The listing builds one solid part. Answer for the finished solid, in the listing's coordinates (mm). A direction names the side the tool comes from. Give positions to 0.01 mm unless a question says otherwise; leave off trailing zeros. Loops run counter-clockwise (first coordinate to the right, second up) from the corner with the lowest first, then second, coordinate; pieces in that order, holes last. Notation, with made-up numbers: M -17,-36.75 L 8,-36.75 A6 ccw 8,-25.75 Z; hole C 88,-34.5 d7. An arc over 180 degrees is marked long. Return JSON: item names as keys, results as strings.
from build123d import *

# Parameters (mm, degrees)
BOSS_EXTRUDE1_DEPTH       = 5.5
SKETCH3_R                 = 4
BOSS_EXTRUDE2_DEPTH       = 5
CHAMFER1_SIZE             = 1
M6X1_0_TAPPED_HOLE1_D     = 5
M6X1_0_TAPPED_HOLE1_DEPTH = 8
M6X1_0_TAPPED_HOLE1_TIP   = 1.502151548


with BuildPart() as part:
    # Sketch1 → Boss-Extrude1 (new, symmetric)
    with BuildSketch(Plane(origin=(0, 0, 0), x_dir=(1, 0, 0), z_dir=(0, 1, 0))):
        Polygon((0, 5.5), (-4.763139721, 2.75), (-4.763139721, -2.75), (0, -5.5), (4.763139721, -2.75), (4.763139721, 2.75), align=None)
    extrude(amount=BOSS_EXTRUDE1_DEPTH, both=True)

    # Sketch3 → Boss-Extrude2 (add)
    with BuildSketch(Plane(origin=(0, 5.5, 0), x_dir=(1, 0, 0), z_dir=(0, 1, 0))):
        with Locations(Location((0, 0, 0), (0, 0, 270))):
            Circle(SKETCH3_R)
    extrude(amount=BOSS_EXTRUDE2_DEPTH)

    # Chamfer1
    chamfer1_edges = [part.edges().sort_by_distance(p)[0] for p in [
        (0, 10.5, -4),
    ]]
    chamfer(chamfer1_edges, length=CHAMFER1_SIZE)

    # M6x1.0 Tapped Hole1
    with Locations(Plane(origin=(0, -5.5, 0), x_dir=(-1, 0, 0), z_dir=(0, -1, 0))):
        with Locations((-0.001364709, 0)):
            Hole(M6X1_0_TAPPED_HOLE1_D / 2, depth=M6X1_0_TAPPED_HOLE1_DEPTH)
            with Locations((0, 0, -(M6X1_0_TAPPED_HOLE1_DEPTH + M6X1_0_TAPPED_HOLE1_TIP / 2))):  # 118° drill point
                Cone(0, M6X1_0_TAPPED_HOLE1_D / 2, M6X1_0_TAPPED_HOLE1_TIP, mode=Mode.SUBTRACT)


solid = part.part
(1) Determine the mould class of faces 3 (the flat face through (-2.348, 0.077, -4.144)), 4 (the cylindrical face through (-3.905, 7.472, -0.867)), 5 (the flat face through (4.763, 0, 0)), 6 (the cylindrical face through (-2.496, -1.444, -0.11)) for opening direction Z: released by +Z, released by -Z, zero draft, split by the parting line, or undercut.
Values follow:
{"face 3": "released by -Z", "face 4": "split by the parting line", "face 5": "zero draft", "face 6": "undercut"}
(2) Straight lines are drawn through the part: line 1 along Y through (x, z) = (1.5, -4.5); line 2 along Z through (x, y) = (-0.75, -0.75); line 3 along X through (y, z) = (1.5, -1). For each, find the intervals that lie inside material, in ascending order.
Values follow:
{"line 1": "-5.5 to 5.5", "line 2": "-5.07 to -2.38, 2.38 to 5.07", "line 3": "-4.76 to -2.29, 2.29 to 4.76"}
(3) The part is cut by section A-A (y = 0.25). Determine the outline of the cut face in (x, z), and give its area (3 significant figures).
Values follow:
{"outline": "M -4.76,-2.75 L 0,-5.5 L 4.76,-2.75 L 4.76,2.75 L 0,5.5 L -4.76,2.75 Z; hole C 0,0 d5", "area": "59.0 mm²"}
(4) The part is cut by section B-B (y = 5.75). Determine the outline of the cut face in (x, z), and give its area (3 significant figures).
Values follow:
{"outline": "C 0,0 d8", "area": "50.3 mm²"}
(5) A tool of negligible diameter and unlimited length cuts with its end or side. For faces 1 (the flat face through (0, -5.5, -3)), 2 (the flat face through (2, 5.5, 4)), from which of +Z, -Z, +X, -X, +Y, -Y can it reach the whole face along a straight path? Write none if from no direction.
Values follow:
{"face 1": "+Z, -Z, +X, -X, -Y", "face 2": "+Y"}
(6) Given pin 1 (1.5 mm diameter, centred on x = 3.5, y = 5.5, fed in from +Z); pin 2 (3 mm diameter, centred on x = 3.5, y = -3, fed in from +Z); pin 3 (4 mm diameter, centred on x = 0, z = 0, fed in from -Y), each flat-ended and moving along its own axis, determine where each tip first touches the part or whether it passes through.
Values follow:
{"pin 1": "z = 3.91", "pin 2": "z = 4.35", "pin 3": "y = 2.8"}
